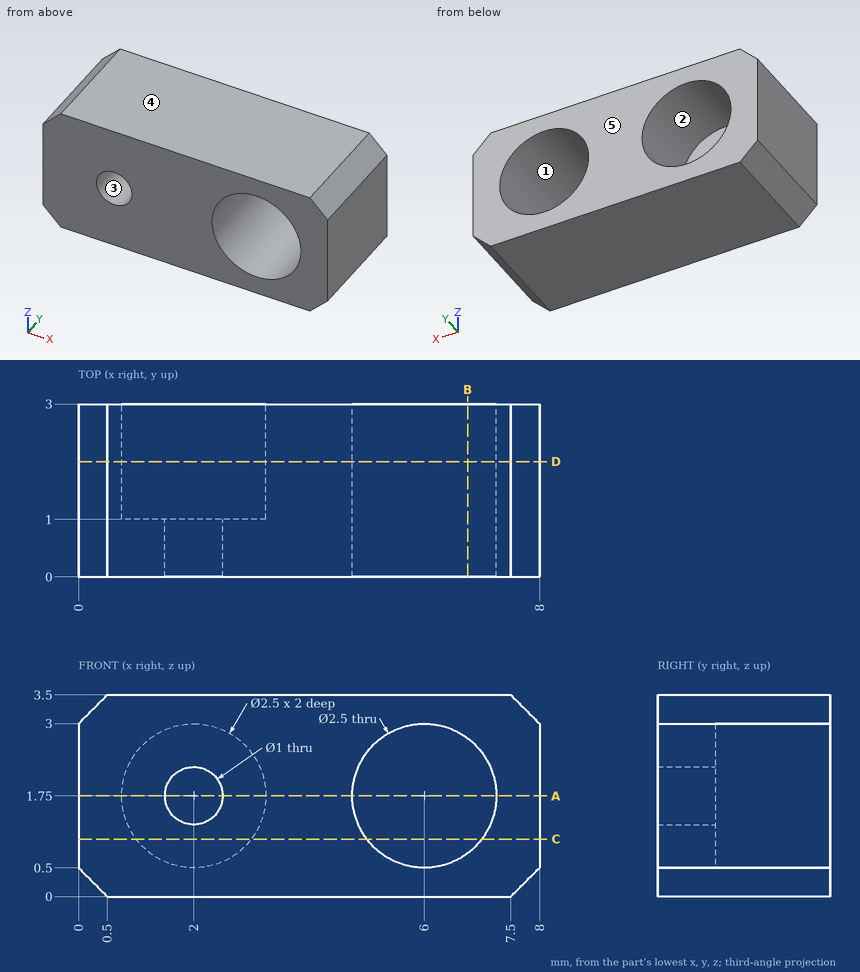
Job drawing, mm, ordinate dimensions from the low corner. One solid piece. A direction names the side the tool comes from. Round coordinates to 2 decimals unless told otherwise and drop trailing zeros. Write each loop counter-clockwise with the first axis right and the second up, starting at its lowest first coordinate (ties: lowest second). Pieces come first, ordered by that corner, then holes.
1) Band-saw the part on D-D, the plane y = 2. List the corners of the cut face in (x, z).
2) 3-axis set-ups, long thin cutter, end or side, ignore diameter. For the marked faces 1 and 2: which of +Z, -Z, +X, -X, +Y, -Y reach the whole face in a straight line?
3) Band-saw the part on B-B, the plane x = 6.75. List the corners of the cut face in (y, z).
4) Mould opens along Z. For the marked faces 3, 4 and 5 say: +Z half, -Z half, draft (parallel to the pull), parting line (faces both ways), or undercut.
5) Band-saw the part on A-A, the plane z = 1.75. List the corners of the cut face in (x, y), and give its area (3 significant figures).
6) Band-saw the part on C-C, the plane z = 1. List the corners of the cut face in (x, y), and give its area (3 significant figures).
7) Drill centre lines: probe 1 along Z at (x, y) = (5, 0.4); probe 2 along Z at (x, y) = (6, 2.15); probe 3 along X at (y, z) = (1.4, 1.95). Where is each one in solid material? Low to high.
Ans:
1. outline: (0, 0.5) - (0.5, 0) - (7.5, 0) - (8, 0.5) - (8, 3) - (7.5, 3.5) - (0.5, 3.5) - (0, 3) - close; hole circle Ø2.5 at (2, 1.75); hole circle Ø2.5 at (6, 1.75)
2. face 1: +Y, -Y
2. face 2: +Y
3. outline: (0, 0) - (3, 0) - (3, 0.75) - (0, 0.75) - close; (0, 2.75) - (3, 2.75) - (3, 3.5) - (0, 3.5) - close
4. face 3: undercut
4. face 4: +Z half
4. face 5: draft
5. outline: (0, 0) - (1.5, 0) - (1.5, 1) - (0.75, 1) - (0.75, 3) - (0, 3) - close; (2.5, 0) - (4.75, 0) - (4.75, 3) - (3.25, 3) - (3.25, 1) - (2.5, 1) - close; (7.25, 0) - (8, 0) - (8, 3) - (7.25, 3) - close
5. area: 10.5 mm2
6. outline: (0, 0) - (5, 0) - (5, 3) - (3, 3) - (3, 1) - (1, 1) - (1, 3) - (0, 3) - close; (7, 0) - (8, 0) - (8, 3) - (7, 3) - close
6. area: 14.0 mm2
7. probe 1: z = 0 to 1, 2.5 to 3.5
7. probe 2: z = 0 to 0.5, 3 to 3.5
7. probe 3: x = 0 to 0.77, 3.23 to 4.77, 7.23 to 8
